from build123d import *

# Parameters (mm, degrees)
SKETCH_1_W          = 68.51
SKETCH_1_H          = 46
EXTRUDE_1_DEPTH     = 23.69
CUT_EXTRUDE_1_REACH = 78.147
CUT_EXTRUDE_2_REACH = 72.493
CUT_EXTRUDE_3_REACH = 60.281
SKETCH_5_W          = 3.5
SKETCH_5_H          = 21
SKETCH_5_W_2        = 44.01
SKETCH_5_H_2        = 39
CUT_EXTRUDE_4_REACH = 59.946
SKETCH_6_R          = 4.5
CUT_EXTRUDE_5_REACH = 72.493
SKETCH_9_R          = 1.45
SKETCH_11_R         = 2.5
CUT_EXTRUDE_6_DEPTH = 3


with BuildPart() as part:
    # 草图1 → 凸台-拉伸1 (new body)
    with BuildSketch(Plane.XY):
        with Locations((-13.62, -0.3125)):
            Rectangle(SKETCH_1_W, SKETCH_1_H)
    extrude(amount=EXTRUDE_1_DEPTH)

    # 草图3 → 切除-拉伸1 (cut, up to next)
    with BuildSketch(Plane(origin=(20.635, 0, 0), x_dir=(0, 0, -1), z_dir=(1, 0, 0)), mode=Mode.PRIVATE) as cut_extrude_1_sk1:
        with BuildLine():
            Line((0, -18.1125), (-16.69, -18.1125))
            ThreePointArc((-16.69, -18.1125), (-19.49, -15.3125), (-16.69, -12.5125))
            Line((-16.69, -12.5125), (0, -12.5125))
            Line((0, -12.5125), (0, -18.1125))
        make_face()
    cut_extrude_1_tool1 = extrude(cut_extrude_1_sk1.sketch, amount=-CUT_EXTRUDE_1_REACH, mode=Mode.PRIVATE) & part.part
    add(cut_extrude_1_tool1.solids().sort_by_distance((20.635, -15.3125, 9.454896))[0], mode=Mode.SUBTRACT)

    # 草图4 → 切除-拉伸2 (cut, up to next)
    with BuildSketch(Plane(origin=(0, 22.6875, 0), x_dir=(1, 0, 0), z_dir=(0, 1, 0)), mode=Mode.PRIVATE) as cut_extrude_2_sk1:
        Polygon((20.635, -23.69), (20.635, -20.89), (17.135, -20.89), (-3.865, -23.69), align=None)
    cut_extrude_2_tool1 = extrude(cut_extrude_2_sk1.sketch, amount=-CUT_EXTRUDE_2_REACH, mode=Mode.PRIVATE) & part.part
    # 草图4 → 切除-拉伸2 (cut, up to next)
    with BuildSketch(Plane(origin=(0, 22.6875, 0), x_dir=(1, 0, 0), z_dir=(0, 1, 0)), mode=Mode.PRIVATE) as cut_extrude_2_sk2:
        Polygon((-47.875, 0), (-47.875, -1.7), (-3.875, -1.7), (8.925, 0), align=None)
    cut_extrude_2_tool2 = extrude(cut_extrude_2_sk2.sketch, amount=-CUT_EXTRUDE_2_REACH, mode=Mode.PRIVATE) & part.part
    add(cut_extrude_2_tool1.solids().sort_by_distance((12.3225, 22.6875, 22.64))[0], mode=Mode.SUBTRACT)
    add(cut_extrude_2_tool2.solids().sort_by_distance((-22.53955, 22.6875, 0.814021))[0], mode=Mode.SUBTRACT)

    # 草图5 → 切除-拉伸3 (cut, up to next)
    with BuildSketch(Plane.XY.offset(23.69), mode=Mode.PRIVATE) as cut_extrude_3_sk1:
        with Locations((18.885, -12.8125)):
            Rectangle(SKETCH_5_W, SKETCH_5_H)
    cut_extrude_3_tool1 = extrude(cut_extrude_3_sk1.sketch, amount=-CUT_EXTRUDE_3_REACH, mode=Mode.PRIVATE) & part.part
    # 草图5 → 切除-拉伸3 (cut, up to next)
    with BuildSketch(Plane.XY.offset(23.69), mode=Mode.PRIVATE) as cut_extrude_3_sk2:
        with Locations((18.885, 12.1875)):
            Rectangle(SKETCH_5_W, SKETCH_5_H)
    cut_extrude_3_tool2 = extrude(cut_extrude_3_sk2.sketch, amount=-CUT_EXTRUDE_3_REACH, mode=Mode.PRIVATE) & part.part
    # 草图5 → 切除-拉伸3 (cut, up to next)
    with BuildSketch(Plane.XY.offset(23.69), mode=Mode.PRIVATE) as cut_extrude_3_sk3:
        with Locations((-25.87, -3.8125)):
            Rectangle(SKETCH_5_W_2, SKETCH_5_H_2)
    cut_extrude_3_tool3 = extrude(cut_extrude_3_sk3.sketch, amount=-CUT_EXTRUDE_3_REACH, mode=Mode.PRIVATE) & part.part
    add(cut_extrude_3_tool1.solids().sort_by_distance((18.885, -12.8125, 23.69))[0], mode=Mode.SUBTRACT)
    add(cut_extrude_3_tool2.solids().sort_by_distance((18.885, 12.1875, 23.69))[0], mode=Mode.SUBTRACT)
    add(cut_extrude_3_tool3.solids().sort_by_distance((-25.87, -3.8125, 23.69))[0], mode=Mode.SUBTRACT)

    # 切除-拉伸4: up to this plane
    cut_extrude_4_end = Plane(origin=(17.135, -23.3135, 20.89), z_dir=(-0.13216372009101784, 0, -0.9912279006826348))
    # 草图6 → 切除-拉伸4 (cut, up to the surface)
    with BuildSketch(Plane(origin=(0.154700714, 0, 1.164805374), x_dir=(-0.9912954083909877, 0, 0.13165642142692813), z_dir=(-0.13165642142692813, 0, -0.9912954083909877)), mode=Mode.PRIVATE) as cut_extrude_4_sk1:
        with Locations((-2.755002186, 0.6875)):
            Circle(SKETCH_6_R)
    cut_extrude_4_tool1 = split(extrude(cut_extrude_4_sk1.sketch, amount=-CUT_EXTRUDE_4_REACH, mode=Mode.PRIVATE), bisect_by=cut_extrude_4_end, keep=Keep.BOTH, mode=Mode.PRIVATE)
    add(cut_extrude_4_tool1.solids().sort_by_distance((2.885722, 0.6875, 0.802092))[0], mode=Mode.SUBTRACT)

    # 草图9 → 切除-拉伸5 (cut, up to next)
    with BuildSketch(Plane(origin=(0, 22.6875, 0), x_dir=(1, 0, 0), z_dir=(0, 1, 0)), mode=Mode.PRIVATE) as cut_extrude_5_sk1:
        with Locations(Location((-25.375, -6.69, 0), (0, 0, 270))):
            Circle(SKETCH_9_R)
    cut_extrude_5_tool1 = extrude(cut_extrude_5_sk1.sketch, amount=-CUT_EXTRUDE_5_REACH, mode=Mode.PRIVATE) & part.part
    # 草图9 → 切除-拉伸5 (cut, up to next)
    with BuildSketch(Plane(origin=(0, 22.6875, 0), x_dir=(1, 0, 0), z_dir=(0, 1, 0)), mode=Mode.PRIVATE) as cut_extrude_5_sk2:
        with Locations(Location((-25.375, -18.69, 0), (0, 0, 270))):
            Circle(SKETCH_9_R)
    cut_extrude_5_tool2 = extrude(cut_extrude_5_sk2.sketch, amount=-CUT_EXTRUDE_5_REACH, mode=Mode.PRIVATE) & part.part
    # 草图9 → 切除-拉伸5 (cut, up to next)
    with BuildSketch(Plane(origin=(0, 22.6875, 0), x_dir=(1, 0, 0), z_dir=(0, 1, 0)), mode=Mode.PRIVATE) as cut_extrude_5_sk3:
        with Locations(Location((-10.375, -18.69, 0), (0, 0, 270))):
            Circle(SKETCH_9_R)
    cut_extrude_5_tool3 = extrude(cut_extrude_5_sk3.sketch, amount=-CUT_EXTRUDE_5_REACH, mode=Mode.PRIVATE) & part.part
    # 草图9 → 切除-拉伸5 (cut, up to next)
    with BuildSketch(Plane(origin=(0, 22.6875, 0), x_dir=(1, 0, 0), z_dir=(0, 1, 0)), mode=Mode.PRIVATE) as cut_extrude_5_sk4:
        with Locations(Location((-10.375, -6.69, 0), (0, 0, 270))):
            Circle(SKETCH_9_R)
    cut_extrude_5_tool4 = extrude(cut_extrude_5_sk4.sketch, amount=-CUT_EXTRUDE_5_REACH, mode=Mode.PRIVATE) & part.part
    add(cut_extrude_5_tool1.solids().sort_by_distance((-25.375, 22.6875, 6.69))[0], mode=Mode.SUBTRACT)
    add(cut_extrude_5_tool2.solids().sort_by_distance((-25.375, 22.6875, 18.69))[0], mode=Mode.SUBTRACT)
    add(cut_extrude_5_tool3.solids().sort_by_distance((-10.375, 22.6875, 18.69))[0], mode=Mode.SUBTRACT)
    add(cut_extrude_5_tool4.solids().sort_by_distance((-10.375, 22.6875, 6.69))[0], mode=Mode.SUBTRACT)

    # 草图11 → 切除-拉伸6 (cut)
    with BuildSketch(Plane(origin=(0, 22.6875, 0), x_dir=(1, 0, 0), z_dir=(0, 1, 0))):
        with Locations(Location((-25.375, -6.69, 0), (0, 0, 270))):
            Circle(SKETCH_11_R)
        with Locations(Location((-10.375, -6.69, 0), (0, 0, 270))):
            Circle(SKETCH_11_R)
        with Locations(Location((-25.375, -18.69, 0), (0, 0, 270))):
            Circle(SKETCH_11_R)
        with Locations(Location((-10.375, -18.69, 0), (0, 0, 270))):
            Circle(SKETCH_11_R)
    extrude(amount=-CUT_EXTRUDE_6_DEPTH, mode=Mode.SUBTRACT)


solid = part.part
Build history of the part. All positions in model axes, mm. A direction names the side the tool comes from. Give positions to 0.01 mm unless a question says otherwise; leave off trailing zeros. Order: outer loops, then holes, each group sorted by start corner. A loop starts at its lowest first (then second) coordinate and runs counter-clockwise, first axis right, second up. Notation, with made-up numbers: M 4,71 L 59,71 A19 cw 59,103 Z; hole C 25.5,25.5 d10. An arc over 180 degrees is marked long. Use one line per item in the form item = value.
Q1. Which spindle directions (+Z, -Z, +X, -X, +Y, -Y) get a long thin tool onto all of the face, cutting with end or side? Do faces 1 (the flat face through (2.44, 5.33, 0.86)), 2 (the flat face through (-3.865, -4, 15)), 3 (the flat face through (-26, 19, 1.7)), 4 (the cylindrical face through (-12.593, 21.208, 19.844)), 5 (the flat face through (-26, 19, 23.69)). Say none if no direction does.
Conclusion:
face_1 = -Z, -X, +Y
face_2 = +Z, -Z, -X, -Y
face_3 = -Z, -X, +Y, -Y
face_4 = +Y
face_5 = +Z, +X, -X, +Y, -Y
Q2. Slice it at C-C, the plane y = -10.5. Write the cut outline in (x, z) (3 decimals).
Conclusion:
outline = M -3.865,1.699 L 8.925,0 L 17.135,0 L 17.135,20.89 L -3.865,23.69 Z
Q3. Slice it at A-A, the plane y = 4.5. Write the cut outline in (x, z) (3 decimals).
Conclusion:
outline = M -3.865,1.699 L 0.516,1.117 L 3.386,22.723 L -3.865,23.69 Z; M 5.255,0.487 L 8.925,0 L 17.135,0 L 17.135,20.89 L 8.125,22.091 Z
Q4. Slice it at B-B, the plane z = 18.69. State how many separate pieces and enclosed holes the cut face has, and give its area (3 significant figures).
Conclusion:
separate_pieces = 4
enclosed_holes = 1
area = 1,090 mm2
Q5. Pull direction Z, two halves, no side cores. Call faces 6 (the flat face through (19, 0, 20.89)), 7 (the flat face through (6, -21, 0)), 8 (the flat face through (17.135, 12, 11)), 9 (the cylindrical face through (-11.26, 17.72, 5.54)): released by +Z, released by -Z, zero draft, split by the parting line, or undercut.
Conclusion:
face_6 = released by +Z
face_7 = released by -Z
face_8 = zero draft
face_9 = undercut
Q6. Wall check: probe 1 along X at (y, z) = (21.9, 18.69) (3 decimals); probe 2 along X at (y, z) = (17.7, 6.69) (3 decimals); probe 3 along Y at (x, z) = (-1.5, 9.5). Give the ranges that are in metal, low to high.
Conclusion:
probe_1 = -47.875 to -27.875, -22.875 to -12.875, -7.875 to 17.135
probe_2 = -47.875 to -26.825, -23.925 to -11.825, -8.925 to 17.135
probe_3 = -23.31 to -18.11, -12.51 to 22.69
Q7. Pin check, flat tips, straight feed: P1, Ø4, axis at y = -18.5, z = 12.5, coming from the -X side (3 decimals); P2, Ø4.5, axis at x = -25.375, z = 18.69, coming from the -Y side; P3, Ø3, axis at x = -10.375, z = 18.69, coming from the +Y side. Stop position of each tip, or through.
Conclusion:
P1 = -3.865
P2 = 15.69
P3 = 19.69
